For this review, take the finished solid that the model builds, in its own axes (mm). A direction names the side the tool comes from. Coordinates: 2 decimals unless noted, no trailing zeros. Write each loop counter-clockwise with the first axis right and the second up, starting at its lowest first coordinate (ties: lowest second). Pieces come first, ordered by that corner, then holes. Notation, with made-up numbers: (55, -24.75) -> (72, -24.75) arc R21 cw to (72, -15.75) -> close; hole circle Ø4 at (6, -13.75). An arc over 180 degrees is marked (long way). Put each result on its own line as item: value. Start each with the question number.
Item 1: Insertion check: P1, Ø10, axis at x = -16.5, z = 32, coming from the -Y side; P2, Ø1.5, axis at y = 7, z = 112, coming from the -X side; P3, Ø1.5, axis at y = 3.5, z = 163.5, coming from the +X side; P4, Ø12, axis at x = -15.5, y = 16.5, coming from the -Z side. Each pin has a flat end and moves straight along its axis. Give the tip position at first contact, or say it passes through.
Item 2: The part is to be moulded in two halves that separate along X. For faces 1 (the cylindrical face through (23.444, 1.201, 145.815)), 2 (the conical face through (13.896, 21.796, 276.86)), 3 (the cylindrical face through (-12, 0, 5)), say which applies: +X half, -X half, draft (parallel to the pull), parting line (faces both ways), or undercut.
Item 3: Consider section A-A on z = 18.5. Give the boundary of the cut face in (x, y).
Item 4: To check wall thickness, follow L1, parallel to Z at x = 23, y = 0; L2, parallel to Y at x = 2, z = 113.5; L3, parallel to X at y = -9, z = 17. State the ranges of each line that lie inside material, in increasing order.
Item 5: For faces 4 (the flat face through (0, 0, 277)), 5 (the cylindrical face through (18, 0, 5)), list the 3-axis set-ups (+Z, -Z, +X, -X, +Y, -Y) from which the entire face can be reached by the end or side of a thin tool; tool diameter is ignored.
```python
from build123d import *

# Parameters (mm, degrees)
SKETCH_1_R      = 27.5
EXTRUDE_1_DEPTH = 277
MM_1_D          = 6
MM_1_DEPTH      = 10
MM_1_TIP        = 1.802581857
MM_2_D          = 8
MM_2_DEPTH      = 8
MM_2_TIP        = 2.403442476
CHAMFER_1_SIZE  = 1.5
CHAMFER_2_SIZE  = 3
CHAMFER_2_SIZE2 = 1.732050808
FILLET_1_R      = 0.5


with BuildPart() as part:
    # 草图1 → 凸台-拉伸1 (new body)
    with BuildSketch(Plane.XY):
        Circle(SKETCH_1_R)
    extrude(amount=EXTRUDE_1_DEPTH)

    # 大小mm 暗销孔1
    with Locations(Plane(origin=(0, 0, 0), x_dir=(1, 0, 0), z_dir=(0, 0, -1))):
        with Locations((15, 0), (-15, 0)):
            Hole(MM_1_D / 2, depth=MM_1_DEPTH)
            with Locations((0, 0, -(MM_1_DEPTH + MM_1_TIP / 2))):  # 118° drill point
                Cone(0, MM_1_D / 2, MM_1_TIP, mode=Mode.SUBTRACT)

    # 大小mm 暗销孔2
    with Locations(Plane(origin=(27.5, 0, 0), x_dir=(0, 0, -1), z_dir=(1, 0, 0))):
        with Locations((-142, 0)):
            Hole(MM_2_D / 2, depth=MM_2_DEPTH)
            with Locations((0, 0, -(MM_2_DEPTH + MM_2_TIP / 2))):  # 118° drill point
                Cone(0, MM_2_D / 2, MM_2_TIP, mode=Mode.SUBTRACT)

    # 倒角1
    chamfer_1_edges = [part.edges().sort_by_distance(p)[0] for p in [
        (-27.5, 0, 0),
    ]]
    chamfer(chamfer_1_edges, length=CHAMFER_1_SIZE)

    # 倒角2
    chamfer_2_edges = [part.edges().sort_by_distance(p)[0] for p in [
        (-27.5, 0, 277),
    ]]
    chamfer_2_side = [part.faces().sort_by_distance(p)[0] for p in [
        (-27.5, 0, 139.25),
    ]]
    chamfer(chamfer_2_edges, length=CHAMFER_2_SIZE, length2=CHAMFER_2_SIZE2, reference=chamfer_2_side[0])

    # 圆角1
    fillet_1_edges = [part.edges().sort_by_distance(p)[0] for p in [
        (-27.5, 0, 274),
    ]]
    fillet(fillet_1_edges, radius=FILLET_1_R)


solid = part.part
```
Return value:
1. P1: y = -24.98
1. P2: x = -26.78
1. P3: x = 27.36
1. P4: z = 0
2. face 1: draft
2. face 2: parting line
2. face 3: undercut
3. outline: circle Ø55 at (0, 0)
4. L1: 0 to 138, 146 to 277
4. L2: -27.43 to 27.43
4. L3: -25.99 to 25.99
5. face 4: +Z, +X, -X, +Y, -Y
5. face 5: -Z
